from build123d import *

# Parameters (mm, degrees)
SKETCH1_R                  = 45
SKETCH1_R_2                = 27.7
BOSS_EXTRUDE1_DEPTH        = 34
F_13_0_13_DIAMETER_HOLE1_D = 13
CHAMFER1_SIZE              = 2


with BuildPart() as part:
    # Sketch1 → Boss-Extrude1 (new body)
    with BuildSketch(Plane.XY):
        Circle(SKETCH1_R)
        Circle(SKETCH1_R_2, mode=Mode.SUBTRACT)
    extrude(amount=BOSS_EXTRUDE1_DEPTH)

    # Ø13.0 (13) Diameter Hole1 (through all)
    with Locations(Plane(origin=(21.131064714, 39.730065493, 17), x_dir=(0.882890344282, -0.469579215865, 0), z_dir=(0.469579215865, 0.882890344282, 0))):
        with Locations((0, 0)):
            Hole(F_13_0_13_DIAMETER_HOLE1_D / 2)

    # Chamfer1
    chamfer1_edges = [part.edges().sort_by_distance(p)[0] for p in [
        (-45, 0, 0),
        (-45, 0, 34),
        (-27.7, 0, 0),
        (-27.7, 0, 34),
    ]]
    chamfer(chamfer1_edges, length=CHAMFER1_SIZE)


solid = part.part
Read the model definition and answer for the solid it produces. Units are mm, in the model's axes. Give positions to 0.01 mm unless a question says otherwise; leave off trailing zeros. Loops run counter-clockwise (first coordinate to the right, second up) from the corner with the lowest first, then second, coordinate; pieces in that order, holes last. Notation, with made-up numbers: (28, 37.5) - (32, 37.5) arc R29 cw to (32, 68.5) - close; hole circle Ø8 at (68, 39). An arc over 180 degrees is marked (long way). Answer as CSV lines item,"result". Start each with the question number.
1) Each of these flat-tipped pins is pushed along its axis until it touches: pin 1 Ø1.5 at (x, z) = (34, 12) entering from -Y; pin 2 Ø4 at (x, z) = (-11.5, 27) entering from -Y; pin 3 Ø2 at (y, z) = (-17.5, 23.5) entering from +X. Where does it stop, or does it pass through?
2) Determine the mould class of faces 1 (the face through (28.1, 10.2, 34)), 2 (the face through (28.1, 10.2, 0)), 3 (the face through (-22.423, -28.956, 15.048)) for opening direction Z: released by +Z, released by -Z, zero draft, split by the parting line, or undercut.
3) Find section C-C (z = 19). Write down the section's boundary in (x, y).
4) Straight lines are drawn through the part: L1, parallel to Y at x = 0, z = 22.5; L2, parallel to X at y = -1, z = 4; L3, parallel to Y at x = 20.5, z = 2. For each, find the intervals that lie inside material, in ascending order. Write a range as from..to.
5) Find section A-A (x = 0). Write down the section's boundary in (y, z).
6) Find section D-D (z = 30). Write down the section's boundary in (x, y), then the cut area to 3 significant figures.
Findings below:
1,pin 1,"y = -30.32"
1,pin 2,"y = -43.99"
1,pin 3,"x = 41.87"
2,face 1,"released by +Z"
2,face 2,"released by -Z"
2,face 3,"undercut"
3,outline,"(-26.39, -36.45) - (-18.14, -20.93) arc R27.7 cw to (7.22, 26.74) - (15.47, 42.26) arc R45 ccw to start; (-15.47, -42.26) arc R45 ccw to (26.39, 36.45) - (18.14, 20.93) arc R27.7 cw to (-7.22, -26.74) - close"
4,L1,"-45..-27.7, 27.7..45"
4,L2,"-44.99..-27.68, 27.68..44.99"
4,L3,"-40.06..-18.63, 18.63..40.06"
5,outline,"(-45, 2) - (-43, 0) - (-29.7, 0) - (-27.7, 2) - (-27.7, 32) - (-29.7, 34) - (-43, 34) - (-45, 32) - close; (27.7, 2) - (29.7, 0) - (43, 0) - (45, 2) - (45, 32) - (43, 34) - (29.7, 34) - (27.7, 32) - close"
6,outline,"circle Ø90 at (0, 0); hole circle Ø55.4 at (0, 0)"
6,area,"3,950 mm^2"
